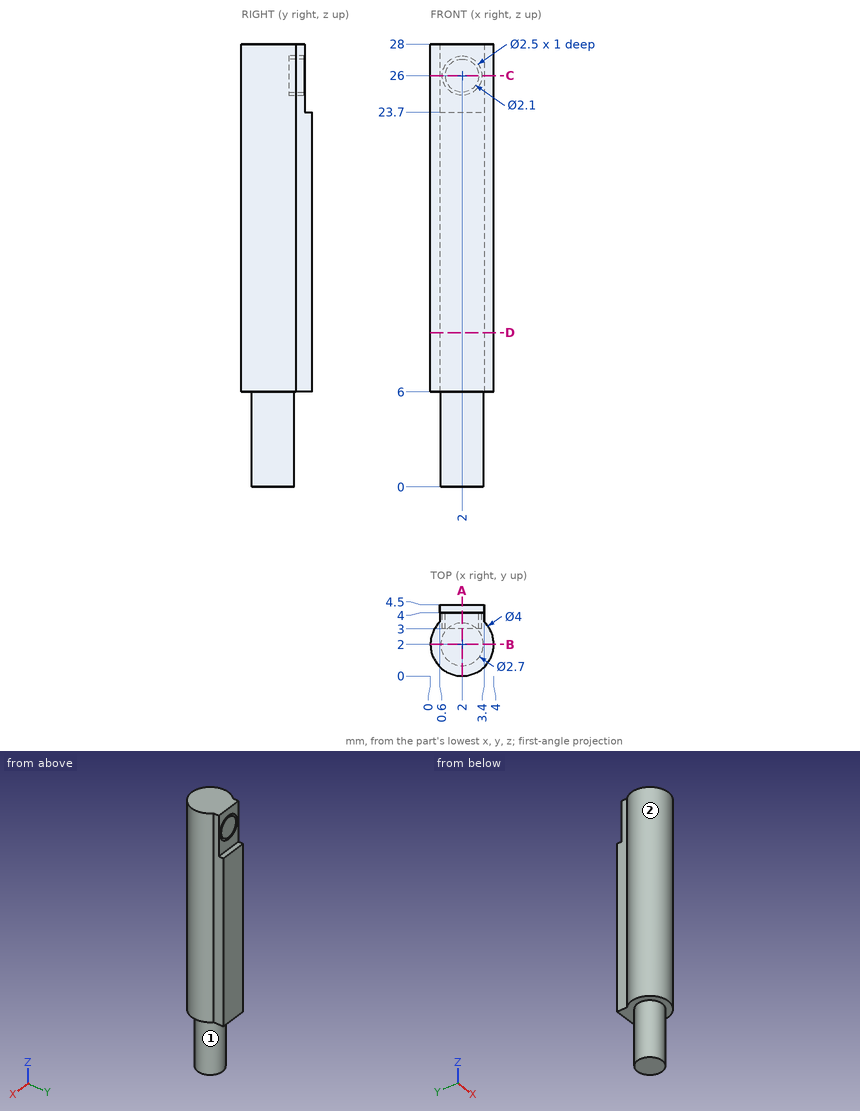
Drawing for the job (mm, zero at the part's lowest x, y, z). A direction names the side the tool comes from. Round coordinates to 2 decimals unless told otherwise and drop trailing zeros. Loops run counter-clockwise (first coordinate to the right, second up) from the corner with the lowest first, then second, coordinate; pieces in that order, holes last. Notation, with made-up numbers: (-40, 39) -> (18, 39) arc R24 cw to (18, 70) -> close; hole circle Ø1 at (-27, 20). An arc over 180 degrees is marked (long way). Answer as CSV lines item,"result". Start each with the question number.
1) Pin check, flat tips, straight feed: P1, Ø2, axis at x = 1.5, z = 26.5, coming from the +Y side; P2, Ø0.9, axis at y = 4, z = 22, coming from the -X side. Stop position of each tip, or through.
2) Probe line 1 along X through (y, z) = (3.45, 26); line 2 along X through (y, z) = (3.2, 26); line 3 along Z through (x, y) = (3.7, 2.3). List the from-to ranges inside material, lowest first.
3) Slice it at D-D (z = 9.75). List the corners of the cut face in (x, y), plus the area to 3 significant figures.
4) Slice it at C-C (z = 26). List the corners of the cut face in (x, y), plus the area to 3 significant figures.
5) Slice it at A-A (x = 2). List the corners of the cut face in (y, z), plus the area to 3 significant figures.
6) Tool access for the marked faces 1 and 2: list every direction of +Z, -Z, +X, -X, +Y, -Y with a clear straight run to the whole face (end or side of a thin tool).
7) Slice it at B-B (y = 2). List the corners of the cut face in (x, z).
Filled in:
1,P1,"stops at y = 4"
1,P2,"stops at x = 0.6"
2,line 1,"x = 0.6 to 0.75, 0.95 to 3.05, 3.25 to 3.4"
2,line 2,"x = 0.4 to 0.75, 0.95 to 3.05, 3.25 to 3.6"
2,line 3,"z = 6 to 28"
3,outline,"(0.6, 3.43) arc R2 ccw (long way) to (3.4, 3.43) -> (3.4, 4.5) -> (0.6, 4.5) -> close"
3,area,"14.5 mm2"
4,outline,"(0.6, 3.43) arc R2 ccw (long way) to (3.4, 3.43) -> (3.4, 4) -> (3.25, 4) -> (3.25, 3) -> (3.05, 3) -> (3.05, 4) -> (0.95, 4) -> (0.95, 3) -> (0.75, 3) -> (0.75, 4) -> (0.6, 4) -> close"
4,area,"12.7 mm2"
5,outline,"(0, 6) -> (0.65, 6) -> (0.65, 0) -> (3.35, 0) -> (3.35, 6) -> (4.5, 6) -> (4.5, 23.7) -> (4, 23.7) -> (4, 24.75) -> (3, 24.75) -> (3, 24.95) -> (4, 24.95) -> (4, 27.05) -> (3, 27.05) -> (3, 27.25) -> (4, 27.25) -> (4, 28) -> (0, 28) -> close"
5,area,"113 mm2"
6,face 1,"-Z"
6,face 2,"+Z, -Z"
7,outline,"(0, 6) -> (0.65, 6) -> (0.65, 0) -> (3.35, 0) -> (3.35, 6) -> (4, 6) -> (4, 28) -> (0, 28) -> close"
